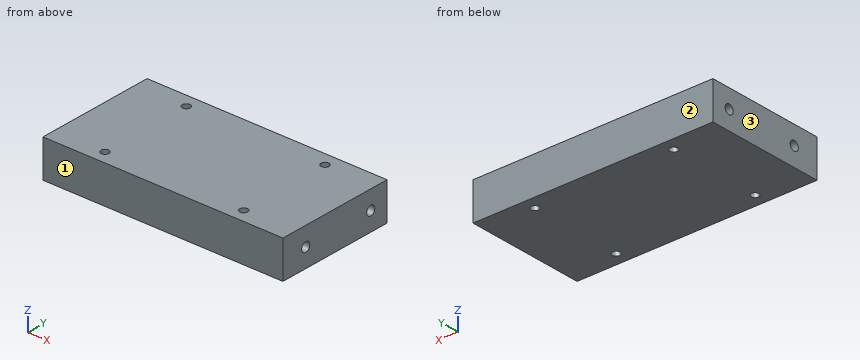
from build123d import *

# Parameters (mm, degrees)
SKETCH_1_W             = 128
SKETCH_1_H             = 64
EXTRUDE_1_DEPTH        = 20
HOLE_WIZARD_M5_1_D     = 4.2
PATTERN_LINEAR_1_COUNT = 2
PATTERN_LINEAR_1_PITCH = 40


with BuildPart() as part:
    # 草图1 → 拉伸1 (new body)
    with BuildSketch(Plane.XY):
        with Locations((64, 32)):
            Rectangle(SKETCH_1_W, SKETCH_1_H)
    extrude(amount=EXTRUDE_1_DEPTH)

    # M5 螺纹孔1 (through all)
    with Locations(Plane.XY.offset(20)):
        with Locations((27, 57), (27, 7), (101, 7), (101, 57)):
            Hole(HOLE_WIZARD_M5_1_D / 2)

    # 草图4 → M5x0.8 螺纹孔1 (revolve, cut)
    with BuildSketch(Plane(origin=(0, 54, 10), x_dir=(0, 0, 1), z_dir=(0, 1, 0))):
        Polygon((0, 0), (0, 18.6618073), (2.1, 17.4), (2.1, 15), (2.5, 15), (2.5, 0), align=None)
    m5x0_8_1 = revolve(axis=Axis((-6.35, 54, 10), (1, 0, 0)), mode=Mode.SUBTRACT)

    # 镜向1: M5x0.8 螺纹孔1 across plane
    add(m5x0_8_1.mirror(Plane(origin=(64, 0, 0), x_dir=(0, 0, 1), z_dir=(1, 0, 0))), mode=Mode.SUBTRACT)

    # 阵列(线性)1: M5x0.8 螺纹孔1 ×2
    with Locations(*[(0, -i * PATTERN_LINEAR_1_PITCH, 0) for i in range(1, PATTERN_LINEAR_1_COUNT)]):
        add(m5x0_8_1, mode=Mode.SUBTRACT)

    # 镜向2 copy 1 sketch → 镜向2 copy 1 (revolve, cut)
    with BuildSketch(Plane(origin=(128, 14, 10), x_dir=(0, 0, 1), z_dir=(0, 1, 0))):
        Polygon((0, 0), (0, -18.6618073), (2.1, -17.4), (2.1, -15), (2.5, -15), (2.5, 0), align=None)
    revolve(axis=Axis((134.35, 14, 10), (1, 0, 0)), mode=Mode.SUBTRACT)

    # 镜向2 copy 2 sketch → 镜向2 copy 2 (revolve, cut)
    with BuildSketch(Plane(origin=(128, 54, 10), x_dir=(0, 0, 1), z_dir=(0, 1, 0))):
        Polygon((0, 0), (0, -18.6618073), (2.1, -17.4), (2.1, -15), (2.5, -15), (2.5, 0), align=None)
    revolve(axis=Axis((134.35, 54, 10), (1, 0, 0)), mode=Mode.SUBTRACT)


solid = part.part
Geometry check sheet. Reference: the model listing, model coordinates, mm. Face numbers are marked on the shaded views. Round coordinates to 2 decimals unless told otherwise and drop trailing zeros. Write each loop counter-clockwise with the first axis right and the second up, starting at its lowest first coordinate (ties: lowest second). Pieces come first, ordered by that corner, then holes. Notation, with made-up numbers: (48.5, 73.5) -> (89.5, 73.5) arc R8 cw to (89.5, 88.5) -> close; hole circle Ø5 at (87, 77.25). An arc over 180 degrees is marked (long way). One line per item, written item: value. Start each with the question number.
(1) Cross-section at A-A, the plane y = 7. Record the cut outline in (x, z), and give its area (3 significant figures).
(2) Draft check along Y on the marked faces 1, 2 and 3. Enter one of: +Y half, -Y half, draft (parallel to the pull), parting line (faces both ways), or undercut.
(3) Cross-section at B-B, the plane x = 27. Record the cut outline in (y, z).
(4) Go/stop test with flat-tipped pins: pin 1 Ø3 at (y, z) = (54, 10) entering from -X; pin 2 Ø2.5 at (y, z) = (54, 10.5) entering from -X; pin 3 Ø2.5 at (y, z) = (14, 10) entering from -X. Record where each tip stops, or that it passes through.
(5) Scan lines: line 1 (Y direction, x = 120.75, z = 10); line 2 (Z direction, x = 111, y = 14); line 3 (X direction, y = 8, z = 12.75). Record each from-to range of solid material in increasing order. Write a range as [from, to].
Answer:
1. outline: (0, 0) -> (24.9, 0) -> (24.9, 20) -> (0, 20) -> close; (29.1, 0) -> (98.9, 0) -> (98.9, 20) -> (29.1, 20) -> close; (103.1, 0) -> (128, 0) -> (128, 20) -> (103.1, 20) -> close
1. area: 2,390 mm²
2. face 1: -Y half
2. face 2: +Y half
2. face 3: draft
3. outline: (0, 0) -> (4.9, 0) -> (4.9, 20) -> (0, 20) -> close; (9.1, 0) -> (54.9, 0) -> (54.9, 20) -> (9.1, 20) -> close; (59.1, 0) -> (64, 0) -> (64, 20) -> (59.1, 20) -> close
4. pin 1: x = 17.76
4. pin 2: x = 17.61
4. pin 3: x = 17.91
5. line 1: [0, 11.5], [16.5, 51.5], [56.5, 64]
5. line 2: [0, 7.9], [12.1, 20]
5. line 3: [0, 25.15], [28.85, 99.15], [102.85, 128]
